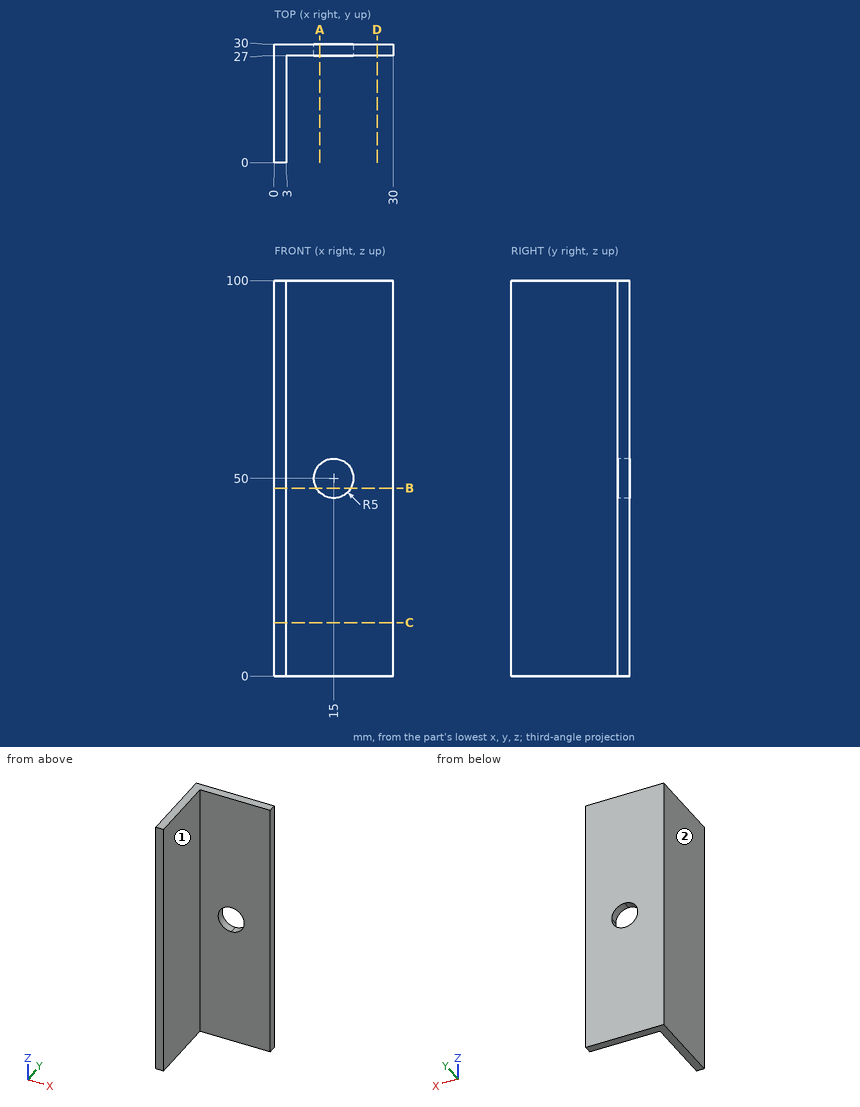
Could you check a few things on this drawing? It's one solid part, dimensions in mm from its lowest x, y, z. A direction names the side the tool comes from. Give positions to 0.01 mm unless a question says otherwise; leave off trailing zeros. Loops run counter-clockwise (first coordinate to the right, second up) from the corner with the lowest first, then second, coordinate; pieces in that order, holes last. Notation, with made-up numbers: M 6,40 L 42,40 A27 cw 42,62 Z; hole C 3.25,72.5 d11. An arc over 180 degrees is marked long. One line per question, with ' | ' between items. Start each with the question number.
Q1. If we section it at C-C (z = 13.5): Please give me the cut outline in (x, y).
Q2. If we section it at D-D (x = 26): Please give me the cut outline in (y, z), plus the area to 3 significant figures.
Q3. If we section it at B-B (z = 47.5): Please give me the cut outline in (x, y), plus the area to 3 significant figures.
Q4. If we section it at A-A (x = 11.5): Please give me the cut outline in (y, z), plus the area to 3 significant figures.
Q5. If I drill on line 1 (Y direction, x = 19.25, z = 8.5); line 2 (X direction, y = 8.5, z = 33), over which ranges is the centre line in solid material (lowest first)? Write a range as from..to.
Q6. For the marked faces 1 and 2, which set-ups out of +Z, -Z, +X, -X, +Y, -Y let a thin tool reach every point of the face, with its end or its side?
Q7. For pin 1 Ø5 at (y, z) = (16.5, 85.5) entering from +X; pin 2 Ø4 at (y, z) = (11, 30.5) entering from -X; pin 3 Ø13.5 at (x, z) = (18, 59) entering from -Y, each with a flat end and sliding along its axis, tell me the tip position at first contact or that it passes through.
Computed:
1) outline: M 0,0 L 3,0 L 3,27 L 30,27 L 30,30 L 0,30 Z
2) outline: M 27,0 L 30,0 L 30,100 L 27,100 Z | area: 300 mm²
3) outline: M 0,0 L 3,0 L 3,27 L 10.67,27 L 10.67,30 L 0,30 Z; M 19.33,27 L 30,27 L 30,30 L 19.33,30 Z | area: 145 mm²
4) outline: M 27,0 L 30,0 L 30,46.43 L 27,46.43 Z; M 27,53.57 L 30,53.57 L 30,100 L 27,100 Z | area: 279 mm²
5) line 1: y = 27..30 | line 2: x = 0..3
6) face 1: +Z, -Z, +X, -Y | face 2: +Z, -Z, -X, +Y, -Y
7) pin 1: stops at x = 3 | pin 2: stops at x = 0 | pin 3: stops at y = 27
